from build123d import *

# Parameters (mm, degrees)
EXTRUDE_1_DEPTH = 382.5


with BuildPart() as part:
    # 草图1 → 凸台-拉伸1 (new, symmetric)
    with BuildSketch(Plane.XY):
        with BuildLine():
            Line((8.903211102, -30.736506504), (40.131056429, -21.690973006))
            ThreePointArc((40.131056429, -21.690973006), (42.792421792, -21.139798433), (45.507033287, -21.007346764))
            Line((45.507033287, -21.007346764), (424.507453379, -31.992863144))
            ThreePointArc((424.507453379, -31.992863144), (433.726976259, -29.589033052), (440.205262247, -22.602631123))
            Line((440.205262247, -22.602631123), (455.205262247, 7.397368877))
            ThreePointArc((455.205262247, 7.397368877), (454.461063742, 23.937428906), (440, 32))
            Line((440, 32), (0, 32))
            ThreePointArc((0, 32), (-31.682552045, -4.496209063), (8.903211102, -30.736506504))
        make_face()
        with BuildLine():
            Line((0, 30), (440, 30))
            ThreePointArc((440, 30), (452.759762125, 22.885966682), (453.416407865, 8.291796068))
            Line((453.416407865, 8.291796068), (438.416407865, -21.708203932))
            ThreePointArc((438.416407865, -21.708203932), (432.700273169, -27.872676222), (424.56540004, -29.993702774))
            Line((424.56540004, -29.993702774), (45.564979948, -19.008186394))
            ThreePointArc((45.564979948, -19.008186394), (42.54012714, -19.155775396), (39.574605735, -19.769941349))
            Line((39.574605735, -19.769941349), (8.346760408, -28.815474848))
            ThreePointArc((8.346760408, -28.815474848), (-29.702392542, -4.215195996), (0, 30))
        make_face(mode=Mode.SUBTRACT)
    extrude(amount=EXTRUDE_1_DEPTH, both=True)


solid = part.part
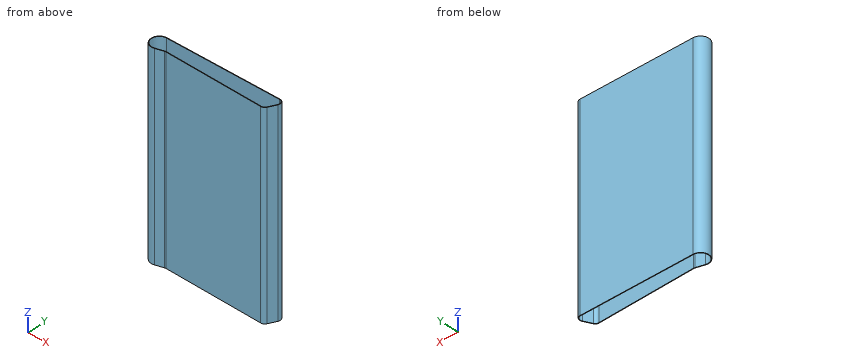
Could you check a few things on this model? Use its own coordinates, in mm. Give positions to 0.01 mm unless a question says otherwise; leave off trailing zeros. Order: outer loops, then holes, each group sorted by start corner. A loop starts at its lowest first (then second) coordinate and runs counter-clockwise, first axis right, second up. Notation, with made-up numbers: (-2, -20) -> (23, -20) arc R27 cw to (23, 16) -> close; hole circle Ø3 at (11, 17). An arc over 180 degrees is marked (long way). Answer in a Markdown table with one row per item. Add a question column.
Item 1: Imagine slicing it at C-C (x = 161.5). List the corners of the cut face in (y, z) for me, and give its area (3 significant figures).
Item 2: I'm going to push flat-ended pins straight in: P1, Ø12, axis at y = -10, z = 288.5, coming from the -X side; P2, Ø1, axis at y = -9, z = 141, coming from the -X side; P3, Ø3, axis at y = -15.5, z = 58, coming from the -X side (3 decimals). Where does each tip first touch, or does it pass through?
Item 3: Please list where these lines run through material, in increasing order: probe 1 along Y at (x, z) = (419, 185.5); probe 2 along X at (y, z) = (24, 252); probe 3 along X at (y, z) = (-7.5, 206.5).
Item 4: Imagine slicing it at A-A (y = 17). List the corners of the cut face in (x, z) for me, and give its area (3 significant figures).
Item 5: Imagine slicing it at B-B (z = -313). List the corners of the cut face in (x, y) for me.
Result:
| question | item | result |
|---|---|---|
| 1 | outline | (-24.37, -382.5) -> (-22.37, -382.5) -> (-22.37, 382.5) -> (-24.37, 382.5) -> close; (30, -382.5) -> (32, -382.5) -> (32, 382.5) -> (30, 382.5) -> close |
| 1 | area | 3,060 mm2 |
| 2 | P1 | x = -31.75 |
| 2 | P2 | x = -30.85 |
| 2 | P3 | x = -28.775 |
| 3 | probe 1 | -31.83 to -29.83, 30 to 32 |
| 3 | probe 2 | -21.17 to -18, 452 to 454.42 |
| 3 | probe 3 | -31.11 to -29.05, 445.52 to 447.76 |
| 4 | outline | (-27.11, -382.5) -> (-24.72, -382.5) -> (-24.72, 382.5) -> (-27.11, 382.5) -> close; (454.87, -382.5) -> (456.88, -382.5) -> (456.88, 382.5) -> (454.87, 382.5) -> close |
| 4 | area | 3,370 mm2 |
| 5 | outline | (0, 32) arc R32 ccw (long way) to (8.9, -30.74) -> (40.13, -21.69) arc R17.5 cw to (45.51, -21.01) -> (424.51, -31.99) arc R17 ccw to (440.21, -22.6) -> (455.21, 7.4) arc R17 ccw to (440, 32) -> close; hole (0, 30) arc R30 ccw (long way) to (8.35, -28.82) -> (39.57, -19.77) arc R19.5 cw to (45.56, -19.01) -> (424.57, -29.99) arc R15 ccw to (438.42, -21.71) -> (453.42, 8.29) arc R15 ccw to (440, 30) -> close |
